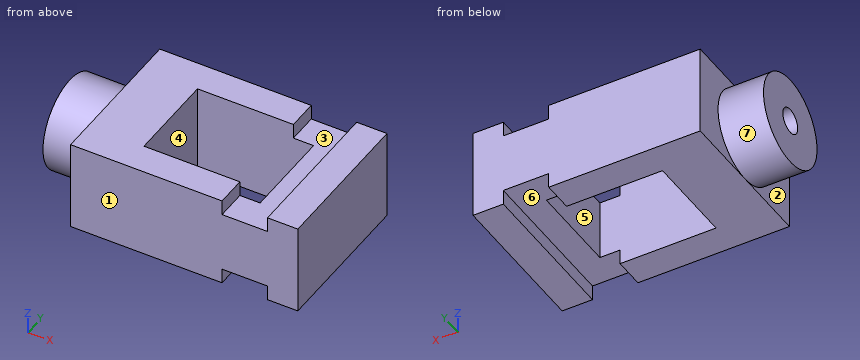
```python
from build123d import *

# Parameters (mm, degrees)
BASE_BLOCK_SKETCH_W        = 90
BASE_BLOCK_SKETCH_H        = 60
BASE_BLOCK_DEPTH           = 36
WINDOW_SKETCH_W            = 46
WINDOW_SKETCH_H            = 36
THROUGH_WINDOW_46X36_DEPTH = 36
BOSS_SKETCH_R              = 18
CYLINDRICAL_BOSS_DEPTH     = 18
BOSS_BORE_SKETCH_R         = 5
BOSS_BORE_DEPTH            = 18
TOP_NOTCHES_SKETCH_W       = 18
TOP_NOTCHES_SKETCH_H       = 6
TOP_NOTCHES_DEPTH          = 95.154128959
END_NOTCH_SKETCH_W         = 18
END_NOTCH_SKETCH_H         = 6
END_NOTCH_DEPTH            = 95.154128959


with BuildPart() as part:
    # Base Block Sketch → Base Block (new body)
    with BuildSketch(Plane.XY):
        Rectangle(BASE_BLOCK_SKETCH_W, BASE_BLOCK_SKETCH_H)
    extrude(amount=BASE_BLOCK_DEPTH)

    # Window Sketch → Through Window 46x36 (cut)
    with BuildSketch(Plane.XY.offset(36)):
        Rectangle(WINDOW_SKETCH_W, WINDOW_SKETCH_H)
    extrude(amount=-THROUGH_WINDOW_46X36_DEPTH, mode=Mode.SUBTRACT)

    # Boss Sketch → Cylindrical Boss (add)
    with BuildSketch(Plane.ZY.offset(45)):
        with Locations((18, 0)):
            Circle(BOSS_SKETCH_R)
    extrude(amount=CYLINDRICAL_BOSS_DEPTH)

    # Boss Bore Sketch → Boss Bore (cut)
    with BuildSketch(Plane.ZY.offset(63)):
        with Locations((18, 0)):
            Circle(BOSS_BORE_SKETCH_R)
    extrude(amount=-BOSS_BORE_DEPTH, mode=Mode.SUBTRACT)

    # Top Notches Sketch → Top Notches (cut, through all)
    with BuildSketch(Plane.XZ.offset(30)):
        with Locations((24, 3)):
            Rectangle(TOP_NOTCHES_SKETCH_W, TOP_NOTCHES_SKETCH_H)
    extrude(amount=-TOP_NOTCHES_DEPTH, mode=Mode.SUBTRACT)

    # End Notch Sketch → End Notch (cut, through all)
    with BuildSketch(Plane.XZ.offset(30)):
        with Locations((24, 33)):
            Rectangle(END_NOTCH_SKETCH_W, END_NOTCH_SKETCH_H)
    extrude(amount=-END_NOTCH_DEPTH, mode=Mode.SUBTRACT)


solid = part.part
```
Work out the finished part from the listing and answer in its coordinate system (mm). Face numbers are marked on the shaded views. A direction names the side the tool comes from. Coordinates: 2 decimals unless noted, no trailing zeros. Loops run counter-clockwise (first coordinate to the right, second up) from the corner with the lowest first, then second, coordinate; pieces in that order, holes last. Notation, with made-up numbers: (29, 41) - (48, 41) arc R13 ccw to (48, 53) - close; hole circle Ø2 at (21, 67). An arc over 180 degrees is marked (long way). Use a Markdown table: item, result.
Item 1: Find section C-C, the plane z = 18. Determine the outline of the cut face in (x, y).
Evaluation:
| item | result |
|---|---|
| outline | (-63, -18) - (-45, -18) - (-45, -30) - (45, -30) - (45, 30) - (-45, 30) - (-45, 18) - (-63, 18) - (-63, 5) - (-45, 5) - (-45, -5) - (-63, -5) - close; hole (-23, -18) - (23, -18) - (23, 18) - (-23, 18) - close |
Item 2: For the marked faces 5, 6 and 7, determine the directions among +Z, -Z, +X, -X, +Y, -Y from which every point of the face is accessible in a straight line to the end or side of a thin tool.
Evaluation:
| item | result |
|---|---|
| face 5 | +Z, -Z |
| face 6 | -Z, +Y, -Y |
| face 7 | -X |
Item 3: Find section D-D, the plane x = 20.5. Determine the outline of the cut face in (y, z).
Evaluation:
| item | result |
|---|---|
| outline | (-30, 6) - (-18, 6) - (-18, 30) - (-30, 30) - close; (18, 6) - (30, 6) - (30, 30) - (18, 30) - close |
Item 4: Find section A-A, the plane x = -18.5. Determine the outline of the cut face in (y, z).
Evaluation:
| item | result |
|---|---|
| outline | (-30, 0) - (-18, 0) - (-18, 36) - (-30, 36) - close; (18, 0) - (30, 0) - (30, 36) - (18, 36) - close |
Item 5: The mould has two halves that part along X. Classify the marked faces 1, 2, 3 and 4: +X half, -X half, draft (parallel to the pull), parting line (faces both ways), or undercut.
Evaluation:
| item | result |
|---|---|
| face 1 | draft |
| face 2 | -X half |
| face 3 | undercut |
| face 4 | undercut |
Item 6: Consider probe 1 along Y at (x, z) = (-57.5, 18); probe 2 along X at (y, z) = (-7, 17); probe 3 along X at (y, z) = (-19, 31). Determine where each line is inside the solid, lowest interval first. Write a range as from..to.
Evaluation:
| item | result |
|---|---|
| probe 1 | y = -18..-5, 5..18 |
| probe 2 | x = -63..-23, 23..45 |
| probe 3 | x = -45..15, 33..45 |
Item 7: Given pin 1 Ø5 at (y, z) = (1, 15.5) entering from -X; pin 2 Ø2 at (y, z) = (-24, 21) entering from -X; pin 3 Ø14.5 at (x, y) = (24, -4) entering from +Z; pin 4 Ø4 at (x, z) = (-52, 15) entering from +Y, each flat-ended and moving along its own axis, determine where each tip first touches the part or whether it passes through.
Evaluation:
| item | result |
|---|---|
| pin 1 | stops at x = -63 |
| pin 2 | stops at x = -45 |
| pin 3 | stops at z = 30 |
| pin 4 | stops at y = 17.97 |
Item 8: Find section B-B, the plane y = 15.5. Determine the outline of the cut face in (x, z).
Evaluation:
| item | result |
|---|---|
| outline | (-63, 8.85) - (-45, 8.85) - (-45, 0) - (-23, 0) - (-23, 36) - (-45, 36) - (-45, 27.15) - (-63, 27.15) - close; (23, 6) - (33, 6) - (33, 0) - (45, 0) - (45, 36) - (33, 36) - (33, 30) - (23, 30) - close |
